```python
from build123d import *

# Parameters (mm, degrees)
SKETCH1_R                    = 152
BOSS_EXTRUDE1_DEPTH          = 50
M14_TAPPED_HOLE1_D           = 12
M14_TAPPED_HOLE1_CSINK_D     = 14.05
M14_TAPPED_HOLE1_CSINK_ANGLE = 90
SKETCH4_R                    = 115
BOSS_EXTRUDE2_DEPTH          = 5
M14_TAPPED_HOLE2_D           = 12
M14_TAPPED_HOLE2_CSINK_D     = 14.05
M14_TAPPED_HOLE2_CSINK_ANGLE = 90
SKETCH8_R                    = 115
CUT_EXTRUDE1_DEPTH           = 222.885105404


with BuildPart() as part:
    # Sketch1 → Boss-Extrude1 (new body)
    with BuildSketch(Plane(origin=(0, 0, 0), x_dir=(1, 0, 0), z_dir=(0, 1, 0))):
        with Locations(Location((0, 0, 0), (0, 0, 270))):
            Circle(SKETCH1_R)
    extrude(amount=BOSS_EXTRUDE1_DEPTH)

    # M14 Tapped Hole1 (through all)
    with Locations(Plane(origin=(0, 50, 0), x_dir=(1, 0, 0), z_dir=(0, 1, 0))):
        with Locations((-68, 117.779454915), (0, 136), (68, 117.779454915), (117.779454915, 68), (136, 0), (117.779454915, -68), (68, -117.779454915), (0, -136), (-68, -117.779454915), (-117.779454915, -68), (-136, 0), (-117.779454915, 68)):
            CounterSinkHole(M14_TAPPED_HOLE1_D / 2, M14_TAPPED_HOLE1_CSINK_D / 2, counter_sink_angle=M14_TAPPED_HOLE1_CSINK_ANGLE)

    # Sketch4 → Boss-Extrude2 (add)
    with BuildSketch(Plane(origin=(0, 50, 0), x_dir=(1, 0, 0), z_dir=(0, 1, 0))):
        with Locations(Location((0, 0, 0), (0, 0, 270))):
            Circle(SKETCH4_R)
    extrude(amount=BOSS_EXTRUDE2_DEPTH)

    # M14 Tapped Hole2 (through all)
    with Locations(Plane(origin=(0, 55, 0), x_dir=(1, 0, 0), z_dir=(0, 1, 0))):
        with Locations((-44, 76.210235533), (0, 88), (44, 76.210235533), (76.210235533, 44), (88, 0), (76.210235533, -44), (44, -76.210235533), (0, -88), (-44, -76.210235533), (-76.210235533, -44), (-88, 0), (-76.210235533, 44)):
            CounterSinkHole(M14_TAPPED_HOLE2_D / 2, M14_TAPPED_HOLE2_CSINK_D / 2, counter_sink_angle=M14_TAPPED_HOLE2_CSINK_ANGLE)

    # Sketch8 → Cut-Extrude1 (cut, through all)
    with BuildSketch(Plane(origin=(0, 55, 0), x_dir=(1, 0, 0), z_dir=(0, 1, 0))):
        with Locations(Location((0, 0, 0), (0, 0, 270))):
            Circle(SKETCH8_R)
    extrude(amount=-CUT_EXTRUDE1_DEPTH, mode=Mode.SUBTRACT)


solid = part.part
```
Here's how the part is built. I have some questions about the finished solid (model axes, mm). Coordinates: 2 decimals unless noted, no trailing zeros. Order: outer loops, then holes, each group sorted by start corner. A loop starts at its lowest first (then second) coordinate and runs counter-clockwise, first axis right, second up.
Item 1: If we section it at C-C, the plane y = 43: Give the number of separate pieces and of enclosed holes in the cut face, then the cut area to 3 significant figures.
Response values:
separate pieces: 1
enclosed holes: 13
area: 29,700 mm2
Item 2: I'm going to push flat-ended pins straight in: pin 1 Ø2 at (y, z) = (41, -107.5) entering from -X; pin 2 Ø4 at (x, y) = (-76, 24.5) entering from +Z; pin 3 Ø9.5 at (x, z) = (-117.78, -68) entering from +Y; pin 4 Ø6 at (x, y) = (-56, 20.5) entering from -Z. Where does each tip first touch, or does it pass through?
Response values:
pin 1: stops at x = -108.45
pin 2: stops at z = 132.77
pin 3: passes through
pin 4: stops at z = -142.46
Item 3: If we section it at B-B, the plane x = 0: List the corners of the cut face in (y, z) for me (3 decimals), then the cut area to 3 significant figures.
Response values:
outline: (0, -152) - (50, -152) - (50, -143.025) - (48.975, -142) - (0, -142) - close; (0, -130) - (48.975, -130) - (50, -128.975) - (50, -115) - (0, -115) - close; (0, 115) - (50, 115) - (50, 128.975) - (48.975, 130) - (0, 130) - close; (0, 142) - (48.975, 142) - (50, 143.025) - (50, 152) - (0, 152) - close
area: 2,500 mm2
Item 4: If we section it at A-A, the plane z = 0: List the corners of the cut face in (x, y) for me (3 decimals), then the cut area to 3 significant figures.
Response values:
outline: (-152, 0) - (-142, 0) - (-142, 48.975) - (-143.025, 50) - (-152, 50) - close; (-130, 0) - (-115, 0) - (-115, 50) - (-128.975, 50) - (-130, 48.975) - close; (115, 0) - (130, 0) - (130, 48.975) - (128.975, 50) - (115, 50) - close; (142, 0) - (152, 0) - (152, 50) - (143.025, 50) - (142, 48.975) - close
area: 2,500 mm2
Item 5: I need wall thicknesses on probe 1 along X at (y, z) = (46, 1); probe 2 along Z at (x, y) = (-62.5, 12); probe 3 along Z at (x, y) = (68, 26.5). Which ranges of each line are inside material? Lowest first, please.
Response values:
probe 1: x = -152 to -141.92, -130.08 to -115, 115 to 130.08, 141.92 to 152
probe 2: z = -138.56 to -120.18, -115.38 to -96.53, 96.53 to 115.38, 120.18 to 138.56
probe 3: z = -135.94 to -123.78, -111.78 to -92.74, 92.74 to 111.78, 123.78 to 135.94
Item 6: If we section it at D-D, the plane z = 40: List the corners of the cut face in (x, y) for me, then the cut area to 3 significant figures.
Response values:
outline: (-146.64, 0) - (-107.82, 0) - (-107.82, 50) - (-146.64, 50) - close; (107.82, 0) - (146.64, 0) - (146.64, 50) - (107.82, 50) - close
area: 3,880 mm2
Item 7: Thinking about a two-plate mould opening in X: for faces 1 (the face through (-66.7, 24.14, -111.92)), 2 (the face through (-92.49, 24.65, -120.62)), 3 (the face through (-112, 50, -34)), which applies, pulls with the +X half, pulls with the -X half, needs draft (parallel to the pull), parting line crosses it, or undercut?
Response values:
face 1: undercut
face 2: parting line crosses it
face 3: needs draft
